The listing builds one solid part. Answer for the finished solid, in the listing's coordinates (mm). Coordinates: 2 decimals unless noted, no trailing zeros. Write each loop counter-clockwise with the first axis right and the second up, starting at its lowest first coordinate (ties: lowest second). Pieces come first, ordered by that corner, then holes. Notation, with made-up numbers: M 69,82 L 76,82 A15 cw 76,92 Z; hole C -34,-35.75 d4. An arc over 180 degrees is marked long. Answer as CSV lines item,"result". Start each with the question number.
```python
from build123d import *

# Parameters (mm, degrees)
CLEARANCE_HOLE_FOR_M1_61_D     = 1.8
CLEARANCE_HOLE_FOR_M1_61_DEPTH = 8
CLEARANCE_HOLE_FOR_M1_61_TIP   = 0.540774557


with BuildPart() as part:
    # Sketch1 → Revolution1 (revolve)
    with BuildSketch(Plane.XY, mode=Mode.PRIVATE) as revolution1_sk:
        with BuildLine():
            Line((0, -37.804295719), (-8, -37.804295719))
            Line((-8, -37.804295719), (-8, 86.695704281))
            ThreePointArc((-8, 86.695704281), (-7.853553391, 87.049257672), (-7.5, 87.195704281))
            Line((-7.5, 87.195704281), (0, 87.195704281))
            Line((0, 87.195704281), (0, -37.804295719))
        make_face()
    revolve(revolution1_sk.sketch.rotate(Axis((0, 38.205391481, 0), (0, -1, 0)), 270), axis=Axis((0, 38.205391481, 0), (0, -1, 0)))

    # Sketch2 → Cut-Revolve1 (revolve, cut)
    with BuildSketch(Plane.XY, mode=Mode.PRIVATE) as cut_revolve1_sk:
        with BuildLine():
            Line((8, 81.81366679), (6.5, 81.81366679))
            ThreePointArc((6.5, 81.81366679), (6.005025253, 81.608641537), (5.8, 81.11366679))
            Line((5.8, 81.11366679), (8, 81.11366679))
            Line((8, 81.11366679), (8, 81.81366679))
        make_face()
        with BuildLine():
            Line((-8, 81.11366679), (-8, 81.81366679))
            Line((-8, 81.81366679), (-6.5, 81.81366679))
            ThreePointArc((-6.5, 81.81366679), (-6.005025253, 81.608641537), (-5.8, 81.11366679))
            Line((-5.8, 81.11366679), (-8, 81.11366679))
        make_face()
    revolve(cut_revolve1_sk.sketch.rotate(Axis((8, 81.11366679, 0), (-1, 0, 0)), 90), axis=Axis((8, 81.11366679, 0), (-1, 0, 0)), mode=Mode.SUBTRACT)

    # Clearance hole for M1.61
    with Locations(Plane(origin=(0, -37.804295719, 0), x_dir=(-1, 0, 0), z_dir=(0, -1, 0))):
        with Locations((0, 0)):
            Hole(CLEARANCE_HOLE_FOR_M1_61_D / 2, depth=CLEARANCE_HOLE_FOR_M1_61_DEPTH)
            with Locations((0, 0, -(CLEARANCE_HOLE_FOR_M1_61_DEPTH + CLEARANCE_HOLE_FOR_M1_61_TIP / 2))):  # 118° drill point
                Cone(0, CLEARANCE_HOLE_FOR_M1_61_D / 2, CLEARANCE_HOLE_FOR_M1_61_TIP, mode=Mode.SUBTRACT)


solid = part.part
```
1) Each of these flat-tipped pins is pushed along its axis until it touches: P1, Ø4, axis at y = 37.5, z = -4, coming from the -X side; P2, Ø2, axis at y = 81.11, z = 0, coming from the -X side; P3, Ø8, axis at x = 4.5, y = -9, coming from the +Z side; P4, Ø5, axis at x = -4.5, y = -12, coming from the +Z side. Where does it stop, or does it pass through?
2) The part is cut by section A-A (y = 70). Determine the outline of the cut face in (x, z), then the cut area to 3 significant figures.
3) Find the intervals of material crossed by line 1 (Y direction, x = -7.45, z = 0); line 2 (X direction, y = 38, z = -5.5); line 3 (Z direction, x = -0.25, y = 54), in increasing order. Write a range as from..to.
Completed:
1,P1,"x = -7.75"
1,P2,"x = -8"
1,P3,"z = 7.98"
1,P4,"z = 7.75"
2,outline,"C 0,0 d16"
2,area,"201 mm²"
3,line 1,"-37.8..80.41, 81.81..87.2"
3,line 2,"-5.81..5.81"
3,line 3,"-8..8"
